Read the model definition and answer for the solid it produces. Units are mm, in the model's axes. A direction names the side the tool comes from. Give positions to 0.01 mm unless a question says otherwise; leave off trailing zeros. Write each loop counter-clockwise with the first axis right and the second up, starting at its lowest first coordinate (ties: lowest second). Pieces come first, ordered by that corner, then holes. Notation, with made-up numbers: M 88,-3 L 131,-3 A24 ccw 131,21 Z; hole C 18,15 d3. An arc over 180 degrees is marked long. Put each result on its own line as item: value.
from build123d import *

# Parameters (mm, degrees)
HUB_HOLES_SKETCH_R = 4
HUB_HOLES_8_DEPTH  = 56.695601263


with BuildPart() as part:
    # Pulley Profile Sketch → Pulley Body (revolve)
    with BuildSketch(Plane.XY):
        Polygon((8, 6), (-8, 6), (-8, 10), (-6, 10), (-6, 29.535898385), (-8, 33), (-8, 41), (-5, 41), (-2.5, 36.669872981), (2.5, 36.669872981), (5, 41), (8, 41), (8, 33), (6, 29.535898385), (6, 10), (8, 10), align=None)
    revolve(axis=Axis((8, 6, 0), (-1, 0, 0)))

    # Hub Holes Sketch → Hub Holes Ø8 (cut, through all)
    with BuildSketch(Plane.ZY.offset(6)):
        with Locations(Location((0, 21.329563784, 0), (0, 0, 270))):
            Circle(HUB_HOLES_SKETCH_R)
        with Locations(Location((-15.329563784, 6, 0), (0, 0, 270))):
            Circle(HUB_HOLES_SKETCH_R)
        with Locations(Location((15.329563784, 6, 0), (0, 0, 270))):
            Circle(HUB_HOLES_SKETCH_R)
        with Locations(Location((0, -9.329563784, 0), (0, 0, 270))):
            Circle(HUB_HOLES_SKETCH_R)
    extrude(amount=-HUB_HOLES_8_DEPTH, mode=Mode.SUBTRACT)


solid = part.part
(1) Which of the six approach directions +Z, -Z, +X, -X, +Y, -Y give full straight-line access (tool end or side, diameter ignored) to faces 1 (the face through (-2.621, -0.694, 30.146)), 2 (the face through (-6, 6, 5)), 3 (the face through (6, 6, 5))?
Result:
face 1: none
face 2: -X
face 3: +X
(2) Section A-A on x = 0.25 is taken. Determine the outline of the cut face in (y, z).
Result:
outline: C 6,0 d61.34; hole C -9.33,0 d8; hole C 6,-15.33 d8; hole C 6,15.33 d8; hole C 21.33,0 d8
(3) Section D-D on x = -7 is taken. Determine the outline of the cut face in (y, z), and give its area (3 significant figures).
Result:
outline: C 6,0 d70; C 6,0 d8; hole C 6,0 d50.54
area: 1,890 mm²
(4) Straight lines are drawn through the part: line 1 along Z through (x, y) = (-0.5, 6); line 2 along Y through (x, z) = (-1.75, -3); line 3 along Y through (x, z) = (-0.5, -3.5). For each, find the intervals that lie inside material, in ascending order. Write a range as from..to.
Result:
line 1: z = -30.67..-19.33, -11.33..11.33, 19.33..30.67
line 2: y = -24.52..-11.98, -6.68..18.68, 23.98..36.52
line 3: y = -24.47..-11.27, -7.39..19.39, 23.27..36.47
(5) For a pull along Z with two mould halves and no side action, classify faces 4 (the face through (-8, -12, 21)), 5 (the face through (7.014, 5.133, 3.905)), 6 (the face through (-6, -22, 21)) as +Z half, -Z half, draft (parallel to the pull), parting line (faces both ways), or undercut.
Result:
face 4: draft
face 5: undercut
face 6: parting line
(6) Given pin 1 Ø3 at (x, z) = (2, 18) entering from -Y; pin 2 Ø23.5 at (y, z) = (7, -7.5) entering from -X; pin 3 Ø13 at (y, z) = (6, -15.33) entering from -X; pin 4 Ø4 at (x, y) = (-5.5, 3) entering from -Z, each flat-ended and moving along its own axis, determine where each tip first touches the part or whether it passes through.
Result:
pin 1: stops at y = -21.1
pin 2: stops at x = -8
pin 3: stops at x = -6
pin 4: stops at z = -34.99
(7) Section B-B on y = 6 is taken. Give the number of separate pieces and of enclosed holes in the cut face, and give its area (3 significant figures).
Result:
separate pieces: 3
enclosed holes: 0
area: 693 mm²
